```python
from build123d import *

# Parameters (mm, degrees)
EXTRUDE_1_DEPTH        = 20
SKETCH_2_R             = 45
CUT_EXTRUDE_1_DEPTH    = 4
SKETCH_3_R             = 19
CUT_EXTRUDE_2_DEPTH    = 104.831594421
SKETCH_4_R             = 35
CUT_EXTRUDE_3_DEPTH    = 4
HOLE_WIZARD_M6_1_D     = 5
HOLE_WIZARD_M6_2_D     = 5
SKETCH_15_W            = 140
SKETCH_15_H            = 120
EXTRUDE_2_DEPTH        = 20
SKETCH_20_W            = 68
SKETCH_20_H            = 120
CUT_EXTRUDE_4_DEPTH    = 2
CHAMFER_1_SIZE         = 10
CHAMFER_2_SIZE         = 60
HOLE_WIZARD_M8_1_D     = 6.8
HOLE_WIZARD_M8_1_DEPTH = 20


with BuildPart() as part:
    # 草图1 → 凸台-拉伸1 (new body)
    with BuildSketch(Plane.XY):
        with BuildLine():
            Line((-70, 0), (-70, 75))
            Line((-70, 75), (70, 75))
            Line((70, 75), (70, 0))
            ThreePointArc((70, 0), (0, -70), (-70, 0))
        make_face()
    extrude(amount=EXTRUDE_1_DEPTH)

    # 草图2 → 切除-拉伸1 (cut)
    with BuildSketch(Plane.XY.offset(20)):
        Circle(SKETCH_2_R)
    extrude(amount=-CUT_EXTRUDE_1_DEPTH, mode=Mode.SUBTRACT)

    # 草图3 → 切除-拉伸2 (cut, through all)
    with BuildSketch(Plane.XY.offset(16)):
        Circle(SKETCH_3_R)
    extrude(amount=-CUT_EXTRUDE_2_DEPTH, mode=Mode.SUBTRACT)

    # 草图4 → 切除-拉伸3 (cut)
    with BuildSketch(Plane(origin=(0, 0, 0), x_dir=(-1, 0, 0), z_dir=(0, 0, -1))):
        Circle(SKETCH_4_R)
    extrude(amount=-CUT_EXTRUDE_3_DEPTH, mode=Mode.SUBTRACT)

    # M6 螺纹孔1 (through all)
    with Locations(Plane.XY.offset(20)):
        with Locations((0, 62.5), (31.25, 54.126587737), (54.126587737, 31.25), (62.5, 0), (54.126587737, -31.25), (31.25, -54.126587737), (0, -62.5), (-31.25, -54.126587737), (-54.126587737, -31.25), (-62.5, 0), (-54.126587737, 31.25), (-31.25, 54.126587737)):
            Hole(HOLE_WIZARD_M6_1_D / 2)

    # M6 螺纹孔2 (through all)
    with Locations(Plane.XY.offset(20)):
        with Locations((0, 0), (31.75, 31.75), (-31.75, -31.75), (-31.75, 31.75), (31.75, -31.75)):
            Hole(HOLE_WIZARD_M6_2_D / 2)

    # 草图15 → 凸台-拉伸2 (add)
    with BuildSketch(Plane(origin=(0, 75, 0), x_dir=(1, 0, 0), z_dir=(0, 1, 0))):
        with Locations((0, -60)):
            Rectangle(SKETCH_15_W, SKETCH_15_H)
    extrude(amount=EXTRUDE_2_DEPTH)

    # 草图20 → 切除-拉伸4 (cut)
    with BuildSketch(Plane(origin=(0, 95, 0), x_dir=(1, 0, 0), z_dir=(0, 1, 0))):
        with Locations((36, -60)):
            Rectangle(SKETCH_20_W, SKETCH_20_H)
    extrude(amount=-CUT_EXTRUDE_4_DEPTH, mode=Mode.SUBTRACT)

    # 倒角1
    chamfer_1_edges = [part.edges().sort_by_distance(p)[0] for p in [
        (70, 84, 120),
    ]]
    chamfer(chamfer_1_edges, length=CHAMFER_1_SIZE)

    # 倒角2
    chamfer_2_edges = [part.edges().sort_by_distance(p)[0] for p in [
        (-70, 85, 120),
    ]]
    chamfer(chamfer_2_edges, length=CHAMFER_2_SIZE)

    # M8 螺纹孔1
    with Locations(Plane(origin=(0, 95, 0), x_dir=(1, 0, 0), z_dir=(0, 1, 0))):
        with Locations((33, -20), (59, -20), (46, -60), (33, -100), (59, -100)):
            Hole(HOLE_WIZARD_M8_1_D / 2, depth=HOLE_WIZARD_M8_1_DEPTH)


solid = part.part
```
Check sheet for the modelled part. Datum: model origin and axes. Units: mm. A direction names the side the tool comes from. Round coordinates to 2 decimals unless told otherwise and drop trailing zeros. Write each loop counter-clockwise with the first axis right and the second up, starting at its lowest first coordinate (ties: lowest second). Pieces come first, ordered by that corner, then holes. Notation, with made-up numbers: M 42.25,-8 L 84.25,-8 A28 cw 84.25,10 Z; hole C 10,76 d10. An arc over 180 degrees is marked long. Write item = value, one per line. Start each with the question number.
1. Tool access check on faces 4 (the flat face through (-0.6, -19.4, 16)), 5 (the cylindrical face through (28, -21, 2)), 6 (the flat face through (-1, 75, 69)), 7 (the cylindrical face through (33.734, -33.271, 9.86)). Record the directions out of +Z, -Z, +X, -X, +Y, -Y that give a thin tool (end or side, any length) a straight path to the whole face; none if there is none.
2. Gauge pin test, flat ends, axial feed: pin 1 (1 mm diameter, centred on y = 94, z = 62, fed in from +X); pin 2 (8 mm diameter, centred on x = 17, y = 18, fed in from +Z); pin 3 (8 mm diameter, centred on x = 31.75, y = -31.75, fed in from +Z); pin 4 (10 mm diameter, centred on x = 37.5, y = 51, fed in from -Z). Record the tip position at first contact, or that the pin passes through.
3. Section check D-D, the plane z = 13. State how many separate pieces and enclosed holes the cut face has, then the cut area to 3 significant figures.
4. Section check C-C, the plane x = -62.5. Record the cut outline in (y, z).
5. Release check for a two-part mould opening along X. For faces 1 (the flat face through (-30, 36, 20)), 2 (the flat face through (70, 77, 31)), 3 (the cylindrical face through (60.19, -0.96, 9.86)) record: pulls with the +X half, pulls with the -X half, needs draft (parallel to the pull), parting line crosses it, or undercut.
6. Section check B-B, the plane y = -16.5. Record the cut outline in (x, z), then the cut area to 3 significant figures.
7. Scan lines: line 1 (X direction, y = 83, z = 100); line 2 (X direction, y = 81, z = 20); line 3 (Y direction, x = 0, z = 7). Record each from-to range of solid material in increasing order. Write a range as [from, to].
8. Section check A-A, the plane z = 32. Record the cut outline in (x, y).
Results found:
q1.face_4 = +Z
q1.face_5 = -Z
q1.face_6 = +Z, +X, -X, -Y
q1.face_7 = +Z, -Z
q2.pin_1 = 2
q2.pin_2 = 16
q2.pin_3 = 20
q2.pin_4 = 0
q3.separate_pieces = 1
q3.enclosed_holes = 17
q3.area = 19,400 mm^2
q4.outline = M -31.52,0 L -2.5,0 L -2.5,20 L -31.52,20 Z; M 2.5,0 L 95,0 L 95,67.5 L 75,67.5 L 75,20 L 2.5,20 Z
q5.face_1 = needs draft
q5.face_2 = pulls with the +X half
q5.face_3 = undercut
q6.outline = M -68.03,0 L -30.87,0 L -30.87,4 L -9.42,4 L -9.42,16 L -41.87,16 L -41.87,20 L -68.03,20 Z; M 9.42,4 L 30.87,4 L 30.87,0 L 68.03,0 L 68.03,20 L 41.87,20 L 41.87,16 L 9.42,16 Z
q6.area = 1,910 mm^2
q7.line_1 = [-30, 29.6], [36.4, 55.6], [62.4, 70]
q7.line_2 = [-70, 29.6], [36.4, 55.6], [62.4, 70]
q7.line_3 = [-70, -65], [-60, -19], [19, 60], [65, 95]
q8.outline = M -70,75 L 70,75 L 70,93 L 2,93 L 2,95 L -70,95 Z
